Check sheet for the modelled part. Datum: model origin and axes. Units: mm. A direction names the side the tool comes from. Round coordinates to 2 decimals unless told otherwise and drop trailing zeros. Order: outer loops, then holes, each group sorted by start corner. A loop starts at its lowest first (then second) coordinate and runs counter-clockwise, first axis right, second up. Notation, with made-up numbers: (45, -13.75) -> (92, -13.75) arc R25 ccw to (92, 11.25) -> close; hole circle Ø11 at (52, 70.25). An arc over 180 degrees is marked (long way). Use CSV: the item, a comma, the result in double quotes.
```python
from build123d import *

# Parameters (mm, degrees)
SKETCH_1_W                     = 296
SKETCH_1_H                     = 62
EXTRUDE_1_DEPTH                = 15
CHAMFER_1_SIZE                 = 10
SKETCH_3_R                     = 22.5
CUT_EXTRUDE_2_DEPTH            = 152.95394039
HOLE_WIZARD_M6_1_D             = 5
SKETCH_6_W                     = 135
SKETCH_6_H                     = 2
CUT_EXTRUDE_3_DEPTH            = 162.161409773
HOLE_WIZARD_M6_1_2_D           = 6.6
HOLE_WIZARD_M6_1_2_CBORE_D     = 11
HOLE_WIZARD_M6_1_2_CBORE_DEPTH = 6.4
HOLE_WIZARD_M8_1_D             = 9
HOLE_WIZARD_M8_1_CBORE_D       = 15
HOLE_WIZARD_M8_1_CBORE_DEPTH   = 8.6
CHAMFER_2_SIZE                 = 0.5


with BuildPart() as part:
    # 草图1 → 凸台-拉伸1 (new body)
    with BuildSketch(Plane.XY):
        Rectangle(SKETCH_1_W, SKETCH_1_H)
    extrude(amount=EXTRUDE_1_DEPTH)

    # 倒角1
    chamfer_1_edges = [part.edges().sort_by_distance(p)[0] for p in [
        (148, -31, 7.5),
        (-148, -31, 7.5),
        (-148, 31, 7.5),
        (148, 31, 7.5),
    ]]
    chamfer(chamfer_1_edges, length=CHAMFER_1_SIZE)

    # 草图3 → 切除-拉伸2 (cut, through all)
    with BuildSketch(Plane(origin=(0, 0, 0), x_dir=(-1, 0, 0), z_dir=(0, 0, -1))):
        Circle(SKETCH_3_R)
    extrude(amount=-CUT_EXTRUDE_2_DEPTH, mode=Mode.SUBTRACT)

    # Hole Wizard M6 _1 (through all)
    with Locations(Plane.XY.offset(15)):
        with Locations((-24, 24), (24, 24), (24, -24), (-24, -24)):
            Hole(HOLE_WIZARD_M6_1_D / 2)

    # 草图6 → 切除-拉伸3 (cut, through all)
    with BuildSketch(Plane.XZ.offset(31)):
        with Locations((0, 1)):
            Rectangle(SKETCH_6_W, SKETCH_6_H)
    extrude(amount=-CUT_EXTRUDE_3_DEPTH, mode=Mode.SUBTRACT)

    # Hole Wizard M6 _1 2 (through all)
    with Locations(Plane.XY.offset(15)):
        with Locations((-47.5, 15), (-61.5, 0), (47.5, 15), (61.5, 0)):
            CounterBoreHole(HOLE_WIZARD_M6_1_2_D / 2, HOLE_WIZARD_M6_1_2_CBORE_D / 2, HOLE_WIZARD_M6_1_2_CBORE_DEPTH)

    # M8 六角凹头螺钉的柱形沉头孔1 (through all)
    with Locations(Plane(origin=(0, 0, 15), x_dir=(-1, 0, 0), z_dir=(0, 0, 1))):
        with Locations((130, 0), (-130, 0)):
            CounterBoreHole(HOLE_WIZARD_M8_1_D / 2, HOLE_WIZARD_M8_1_CBORE_D / 2, HOLE_WIZARD_M8_1_CBORE_DEPTH)

    # 倒角2
    chamfer_2_edges = [part.edges().sort_by_distance(p)[0] for p in [
        (102.75, 31, 0),
        (0, 31, 15),
        (148, 0, 0),
        (-102.75, -31, 0),
        (-148, 0, 0),
        (-143, -26, 0),
        (-143, 26, 0),
        (143, -26, 0),
        (143, 26, 0),
        (148, 0, 15),
        (-148, 0, 15),
        (0, -31, 15),
        (-143, -26, 15),
        (-143, 26, 15),
        (143, -26, 15),
        (143, 26, 15),
        (-102.75, 31, 0),
        (102.75, -31, 0),
        (67.5, 0, 0),
        (-67.5, 0, 0),
    ]]
    chamfer(chamfer_2_edges, length=CHAMFER_2_SIZE)


solid = part.part
```
Q1. Mould release check, pull along Y, two halves, no side actions. Record for faces 1 (the face through (-2, 31, 7)), 2 (the face through (142.756, -25.896, 14.747)), 3 (the face through (-67, 0, 12)): pulls with the +Y half, pulls with the -Y half, needs draft (parallel to the pull), parting line crosses it, or undercut.
Result sheet:
face 1,"pulls with the +Y half"
face 2,"pulls with the -Y half"
face 3,"undercut"
Q2. Sectioned sample at B-B, the plane y = 15. State how many separate pieces and enclosed holes the cut face has, then the cut area to 3 significant figures.
Result sheet:
separate pieces,"4"
enclosed holes,"0"
area,"3,510 mm^2"
Q3. Scan lines: L1, parallel to X at y = -0.5, z = 5.5; L2, parallel to X at y = -4.5, z = 8; L3, parallel to X at y = 1.5, z = 6.75. Record each from-to range of solid material in increasing order.
Result sheet:
L1,"x = -148 to -134.47, -125.53 to -64.76, -58.24 to -22.49, 22.49 to 58.24, 64.76 to 125.53, 134.47 to 148"
L2,"x = -148 to -136, -124 to -22.05, 22.05 to 124, 136 to 148"
L3,"x = -148 to -137.35, -122.65 to -64.44, -58.56 to -22.45, 22.45 to 58.56, 64.44 to 122.65, 137.35 to 148"
Q4. Access from +Z, -Z, +X, -X, +Y, -Y to the whole of each face (thin tool, end or side, straight path). Record for faces 4 (the face through (-135, 0, 6.4)), 5 (the face through (-23.67, 26.48, 8.41)), 6 (the face through (14, -21, 2)).
Result sheet:
face 4,"+Z"
face 5,"+Z, -Z"
face 6,"-Z, +Y, -Y"
Q5. Sectioned sample at C-C, the plane x = -61.5. Enter the section's corners in (y, z), then the cut area to 3 significant figures.
Result sheet:
outline,"(-31, 2) -> (-3.3, 2) -> (-3.3, 8.6) -> (-5.5, 8.6) -> (-5.5, 15) -> (-30.5, 15) -> (-31, 14.5) -> close; (3.3, 2) -> (31, 2) -> (31, 14.5) -> (30.5, 15) -> (5.5, 15) -> (5.5, 8.6) -> (3.3, 8.6) -> close"
area,"692 mm^2"
Q6. Sectioned sample at A-A, the plane x = -130. Enter the section's corners in (y, z), then the cut area to 3 significant figures.
Result sheet:
outline,"(-31, 0.5) -> (-30.5, 0) -> (-4.5, 0) -> (-4.5, 6.4) -> (-7.5, 6.4) -> (-7.5, 15) -> (-30.5, 15) -> (-31, 14.5) -> close; (4.5, 0) -> (30.5, 0) -> (31, 0.5) -> (31, 14.5) -> (30.5, 15) -> (7.5, 15) -> (7.5, 6.4) -> (4.5, 6.4) -> close"
area,"743 mm^2"
Q7. Go/stop test with flat-tipped pins: pin 1 (2 mm diameter, centred on y = 24.5, z = 8.5, fed in from -X); pin 2 (9 mm diameter, centred on x = -47.5, y = 15, fed in from -Z); pin 3 (10.5 mm diameter, centred on x = 61.5, y = 0, fed in from +Z). Record where each tip stops, or that it passes through.
Result sheet:
pin 1,"stops at x = -145.5"
pin 2,"stops at z = 2"
pin 3,"stops at z = 8.6"
